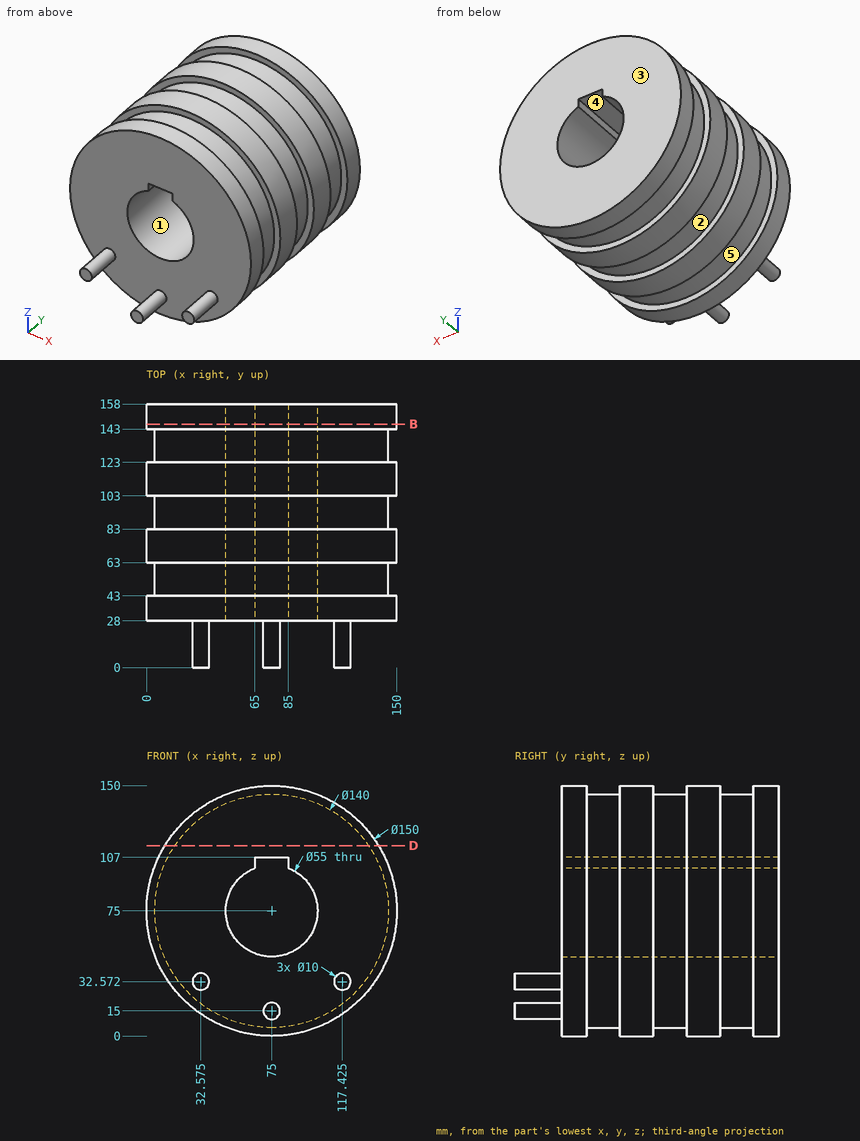
Drawing for the job (mm, zero at the part's lowest x, y, z). A direction names the side the tool comes from. Give positions to 0.01 mm unless a question says otherwise; leave off trailing zeros. Order: outer loops, then holes, each group sorted by start corner. A loop starts at its lowest first (then second) coordinate and runs counter-clockwise, first axis right, second up. Notation, with made-up numbers: M 38,8.5 L 54,8.5 A30 cw 54,38.5 Z; hole C 57.25,-10 d3. An arc over 180 degrees is marked long. Use a Markdown table: item, result. Add a question column.
(1) Saw through at B-B, the plane y = 146. Give the cut face in (x, z), and give its area (3 significant figures).
(2) Mould opens along Z. For the marked faces 1, 2 and 3 say: +Z half, -Z half, draft (parallel to the pull), parting line (faces both ways), or undercut.
(3) Probe line 1 along Y through (x, z) = (49.5, 6.5); line 2 along X through (y, z) = (109, 75); line 3 along Y through (x, z) = (66.5, 143). List the from-to ranges inside material, lowest first. Write a range as [from, to].
(4) Drop flat-ended pins along their axis: P1, Ø3, axis at y = 100.5, z = 104.5, coming from the -X side; P2, Ø10, axis at y = 41, z = 64.5, coming from the +X side; P3, Ø5, axis at y = 89.5, z = 69.5, coming from the +X side. Give the stop position or say it passes through.
(5) Saw through at D-D, the plane z = 114. Give the cut face in (x, y), and give its area (3 significant figures).
(6) 3-axis set-ups, long thin cutter, end or side, ignore diameter. For the marked faces 4 and 5: which of +Z, -Z, +X, -X, +Y, -Y reach the whole face in a straight line?
Answer key:
| question | item | result |
|---|---|---|
| 1 | outline | C 75,75 d150; hole M 65,100.62 A27.5 ccw long 85,100.62 L 85,107 L 65,107 Z |
| 1 | area | 15,200 mm^2 |
| 2 | face 1 | undercut |
| 2 | face 2 | parting line |
| 2 | face 3 | draft |
| 3 | line 1 | [28, 43], [63, 83], [103, 123], [143, 158] |
| 3 | line 2 | [0, 47.5], [102.5, 150] |
| 3 | line 3 | [28, 158] |
| 4 | P1 | x = 10.84 |
| 4 | P2 | x = 149.8 |
| 4 | P3 | x = 144.94 |
| 5 | outline | M 10.94,28 L 139.06,28 L 139.06,43 L 133.13,43 L 133.13,63 L 139.06,63 L 139.06,83 L 133.13,83 L 133.13,103 L 139.06,103 L 139.06,123 L 133.13,123 L 133.13,143 L 139.06,143 L 139.06,158 L 10.94,158 L 10.94,143 L 16.87,143 L 16.87,123 L 10.94,123 L 10.94,103 L 16.87,103 L 16.87,83 L 10.94,83 L 10.94,63 L 16.87,63 L 16.87,43 L 10.94,43 Z |
| 5 | area | 15,900 mm^2 |
| 6 | face 4 | +Y, -Y |
| 6 | face 5 | none |
